from build123d import *

# Parameters (mm, degrees)
EXTRUDE_START       = -16.5
SKETCH_3_R          = 2
EXTRUDE_2_DEPTH     = 16.5
EXTRUDE_START_2     = -5.3
SKETCH_2_R          = 2
EXTRUDE_1_DEPTH     = 5.3
SKETCH_6_R          = 3
CUT_EXTRUDE_1_DEPTH = 10


with BuildPart() as part:
    # 草图1 → 旋转1 (revolve)
    with BuildSketch(Plane.XY, mode=Mode.PRIVATE) as revolve_1_sk:
        with BuildLine():
            Line((0, 2), (0, 4.2))
            Line((0, 4.2), (0.8, 5))
            Line((0.8, 5), (4.7, 5))
            Line((4.7, 5), (5.025001538, 4.674998462))
            ThreePointArc((5.025001538, 4.674998462), (5.539435688, 4.40084215), (6.119340804, 4.460123138))
            Line((6.119340804, 4.460123138), (8, 5.25))
            Line((8, 5.25), (8, 7))
            Line((8, 7), (9, 7))
            Line((9, 7), (14.3, 7))
            Line((14.3, 7), (14.3, 5))
            Line((14.3, 5), (19, 5))
            Line((19, 5), (19, 7.5))
            Line((19, 7.5), (35.5, 7.5))
            Line((35.5, 7.5), (35.5, 3.75))
            Line((35.5, 3.75), (40, 3.75))
            Line((40, 3.75), (40, 2))
            Line((40, 2), (0, 2))
        make_face()
    revolve(revolve_1_sk.sketch.rotate(Axis((0, 0, 0), (1, 0, 0)), 90), axis=Axis((0, 0, 0), (1, 0, 0)))

    # 草图3 → 拉伸2 (add)
    with BuildSketch(Plane(origin=(35.5, 0, 0), x_dir=(0, 0, -1), z_dir=(1, 0, 0)).offset(EXTRUDE_START)):
        Polygon((7.5, -4.330127019), (7.5, 4.330127019), (0, 8.660254038), (-7.5, 4.330127019), (-7.5, -4.330127019), (0, -8.660254038), align=None)
        with Locations(Location((0, 0, 0), (0, 0, 180))):
            Circle(SKETCH_3_R, mode=Mode.SUBTRACT)
    extrude(amount=EXTRUDE_2_DEPTH)

    # 草图2 → 凸台-拉伸1 (add)
    with BuildSketch(Plane(origin=(14.3, 0, 0), x_dir=(0, 0, -1), z_dir=(1, 0, 0)).offset(EXTRUDE_START_2)):
        Polygon((-7, 4.041451884), (-7, -4.041451884), (0, -8.082903769), (7, -4.041451884), (7, 4.041451884), (0, 8.082903769), align=None)
        with Locations(Location((0, 0, 0), (0, 0, 180))):
            Circle(SKETCH_2_R, mode=Mode.SUBTRACT)
    extrude(amount=EXTRUDE_1_DEPTH)

    # 草图4 → 切除-旋转1 (revolve, cut)
    with BuildSketch(Plane.XY):
        Polygon((9, 7), (9.625214782, 8.082903769), (9, 8.082903769), align=None)
        Polygon((14.3, 7), (13.674785218, 8.082903769), (14.3, 8.082903769), align=None)
        Polygon((19, 7.5), (19.669872981, 8.660254038), (19, 8.660254038), align=None)
        Polygon((35.5, 7.5), (34.830127019, 8.660254038), (35.5, 8.660254038), align=None)
    revolve(axis=Axis((0, 0, 0), (1, 0, 0)), mode=Mode.SUBTRACT)

    # 草图6 → 切除-拉伸1 (cut)
    with BuildSketch(Plane(origin=(40, 0, 0), x_dir=(0, 0, -1), z_dir=(1, 0, 0))):
        Circle(SKETCH_6_R)
    extrude(amount=-CUT_EXTRUDE_1_DEPTH, mode=Mode.SUBTRACT)


solid = part.part
Model file for the job. Use its own axes, mm. A direction names the side the tool comes from. Give positions to 0.01 mm unless a question says otherwise; leave off trailing zeros. Loops run counter-clockwise (first coordinate to the right, second up) from the corner with the lowest first, then second, coordinate; pieces in that order, holes last. Notation, with made-up numbers: (48, 16.5) -> (64, 16.5) arc R28 cw to (64, 48.5) -> close; hole circle Ø4 at (-22, 67.5). An arc over 180 degrees is marked (long way). Use a Markdown table: item, result. Add a question column.
(1) Wall check: line 1 along X through (y, z) = (5.75, -2.75); line 2 along Y through (x, z) = (16.75, 0); line 3 along Z through (x, y) = (11, -3). Give the ranges that are in metal, low to high.
(2) Mould opens along X. For faces 4 (the conical face through (35.337, 3.907, 6.73)), 5 (the conical face through (9.15, 3.65, 6.28)), 6 (the flat face through (19, -5, -2)) say: +X half, -X half, draft (parallel to the pull), parting line (faces both ways), or undercut.
(3) Slice it at A-A on x = 25. List the corners of the cut face in (y, z).
(4) Drop flat-ended pins along their axis: pin 1 Ø1.5 at (x, z) = (24, -1) entering from +Y; pin 2 Ø1.6 at (x, y) = (10.5, 1.5) entering from +Z; pin 3 Ø1 at (x, z) = (27.5, -4.5) entering from +Y. Give the stop position or say it passes through.
(5) Tool access for faces 1 (the cylindrical face through (8.51, 6.21, 3.23)), 2 (the cylindrical face through (37.78, -3.16, 2.02)), 3 (the conical face through (19.16, -7.78, 0.02)): list every direction of +Z, -Z, +X, -X, +Y, -Y with a clear straight run to the whole face (end or side of a thin tool).
Filled sheet:
| question | item | result |
|---|---|---|
| 1 | line 1 | 8 to 14.3, 19 to 35.5 |
| 1 | line 2 | -5 to -2, 2 to 5 |
| 1 | line 3 | -7 to 7 |
| 2 | face 4 | +X half |
| 2 | face 5 | -X half |
| 2 | face 6 | undercut |
| 3 | outline | (-8.66, 0) -> (-4.33, -7.5) -> (4.33, -7.5) -> (8.66, 0) -> (4.33, 7.5) -> (-4.33, 7.5) -> close; hole circle Ø4 at (0, 0) |
| 4 | pin 1 | y = 8.52 |
| 4 | pin 2 | z = 7 |
| 4 | pin 3 | y = 6.35 |
| 5 | face 1 | -X |
| 5 | face 2 | +X |
| 5 | face 3 | -Y |
